For this review, take the finished solid that the model builds, in its own axes (mm). A direction names the side the tool comes from. Give positions to 0.01 mm unless a question says otherwise; leave off trailing zeros. Order: outer loops, then holes, each group sorted by start corner. A loop starts at its lowest first (then second) coordinate and runs counter-clockwise, first axis right, second up. Notation, with made-up numbers: (-27, 76.25) - (-9, 76.25) arc R26 cw to (-9, 92.25) - close; hole circle Ø9 at (22.25, -23). An arc over 180 degrees is marked (long way). One line per item, written item: value.
```python
from build123d import *

# Parameters (mm, degrees)
BASE_PLATE_DEPTH                      = 18
BASE_CORNERS_AND_MOUNTING_HOLES_DEPTH = 36
BASE_RELIEF_SKETCH_R                  = 6
BASE_RELIEF_CUT_DEPTH                 = 36
SUPPORT_UPRIGHT_DEPTH                 = 34
UPRIGHT_TAPER_CUT_DEPTH               = 87.764047854
BEARING_SEAT_CUT_DEPTH                = 12


with BuildPart() as part:
    # Base Plate Profile → Base Plate (new, symmetric)
    with BuildSketch(Plane.XY):
        Polygon((0, 0), (50, 0), (50, 12), (-50, 12), (-50, 0), align=None)
    extrude(amount=BASE_PLATE_DEPTH, both=True)

    # Base Corners and Holes Sketch → Base Corners and Mounting Holes (cut)
    with BuildSketch(Plane(origin=(0, 12, 0), x_dir=(1, 0, 0), z_dir=(0, 1, 0))):
        with BuildLine():
            Line((-50, -14), (-50, -18))
            Line((-50, -18), (-46, -18))
            ThreePointArc((-46, -18), (-48.828427125, -16.828427125), (-50, -14))
        make_face()
        with BuildLine():
            Line((50, -14), (50, -18))
            Line((50, -18), (46, -18))
            ThreePointArc((46, -18), (48.828427125, -16.828427125), (50, -14))
        make_face()
        with BuildLine():
            Line((50, 14), (50, 18))
            Line((50, 18), (46, 18))
            ThreePointArc((46, 18), (48.828427125, 16.828427125), (50, 14))
        make_face()
        with BuildLine():
            Line((-50, 18), (-46, 18))
            ThreePointArc((-46, 18), (-48.828427125, 16.828427125), (-50, 14))
            Line((-50, 14), (-50, 18))
        make_face()
    extrude(amount=-BASE_CORNERS_AND_MOUNTING_HOLES_DEPTH, mode=Mode.SUBTRACT)

    # Base Relief Sketch → Base Relief Cut (cut)
    with BuildSketch(Plane(origin=(0, 12, 0), x_dir=(1, 0, 0), z_dir=(0, 1, 0))):
        with Locations(Location((-36, 0, 0), (0, 0, 180))):
            Circle(BASE_RELIEF_SKETCH_R)
        with Locations(Location((36, 0, 0), (0, 0, 270))):
            Circle(BASE_RELIEF_SKETCH_R)
    extrude(amount=-BASE_RELIEF_CUT_DEPTH, mode=Mode.SUBTRACT)

    # Upright Profile → Support Upright (add)
    with BuildSketch(Plane.XY.offset(18)):
        with BuildLine():
            Line((8, 39.150951317), (8, 48))
            Line((8, 48), (20, 48))
            Line((20, 48), (20, 12))
            Line((20, 12), (-20, 12))
            Line((-20, 12), (-20, 48))
            Line((-20, 48), (-8, 48))
            Line((-8, 48), (-8, 39.150951317))
            ThreePointArc((-8, 39.150951317), (0, 31.150951317), (8, 39.150951317))
        make_face()
    extrude(amount=-SUPPORT_UPRIGHT_DEPTH)

    # Upright Taper Sketch → Upright Taper Cut (cut, through all)
    with BuildSketch(Plane.ZY.offset(20)):
        Polygon((-8, 48), (18, 48), (18, 12), (16, 12), align=None)
    extrude(amount=-UPRIGHT_TAPER_CUT_DEPTH, mode=Mode.SUBTRACT)

    # Bearing Seat Sketch → Bearing Seat Cut (cut, symmetric)
    with BuildSketch(Plane(origin=(0, 0, 0), x_dir=(0, 0, -1), z_dir=(1, 0, 0))):
        Polygon((8, 48), (8, 12), (-16, 12), align=None)
    extrude(amount=BEARING_SEAT_CUT_DEPTH, both=True, mode=Mode.SUBTRACT)


solid = part.part
```
(1) Take a section at D-D (z = -12). Write out the cut boundary in (x, y), then the cut area to 3 significant figures.
Answers below:
outline: (-50, 0) - (50, 0) - (50, 12) - (20, 12) - (20, 48) - (8, 48) - (8, 39.15) arc R8 cw to (-8, 39.15) - (-8, 48) - (-20, 48) - (-20, 12) - (-50, 12) - close
area: 2,400 mm^2
(2) For P1, Ø12, axis at y = 38.5, z = 0, coming from the -X side; P2, Ø7, axis at x = 36, z = 0, coming from the +Y side; P3, Ø9, axis at y = 41.5, z = -10, coming from the +X side; P4, Ø1, axis at x = -6, y = 20, coming from the -Z side, all flat-tipped, find the tip position at first contact; note any pin that passes through.
Answers below:
P1: stops at x = -20
P2: passes through
P3: stops at x = 20
P4: stops at z = -16
(3) Take a section at C-C (y = 15). Write out the cut boundary in (x, z), then the cut area to 3 significant figures.
Answers below:
outline: (-20, -16) - (20, -16) - (20, 14) - (12, 14) - (12, -8) - (-12, -8) - (-12, 14) - (-20, 14) - close
area: 672 mm^2
(4) Take a section at B-B (x = 36). Write out the cut boundary in (y, z).
Answers below:
outline: (0, -18) - (12, -18) - (12, -6) - (0, -6) - close; (0, 6) - (12, 6) - (12, 18) - (0, 18) - close
(5) Wall thickness on line 1 (Z direction, x = -36, y = 4); line 2 (X direction, y = 20, z = -7); line 3 (X direction, y = 39.5, z = -12): over which ranges is each line inside the solid? List them lowest first. Write a range as from..to.
Answers below:
line 1: z = -18..-6, 6..18
line 2: x = -20..-12, 12..20
line 3: x = -20..-8, 8..20
(6) Machinability: for faces 1 (the face through (-8, 44, -12)), 2 (the face through (20, 26, -3)), 3 (the face through (-20, 26, -3)), 4 (the face through (12, 22, -2)), 5 (the face through (0, 30, -16)), which of the approach directions +Z, -Z, +X, -X, +Y, -Y give a long, thin tool a straight path to every point of the face, cutting with its end or side? Answer none if there is none.
Answers below:
face 1: +Z, -Z, +Y
face 2: +Z, -Z, +X, +Y
face 3: +Z, -Z, -X, +Y
face 4: +Z, +Y
face 5: -Z, +X, -X, +Y
(7) Take a section at A-A (z = 0). Write out the cut boundary in (x, y), then the cut area to 3 significant figures.
Answers below:
outline: (-50, 0) - (-42, 0) - (-42, 12) - (-50, 12) - close; (-30, 0) - (30, 0) - (30, 12) - (20, 12) - (20, 36) - (12, 36) - (12, 12) - (-12, 12) - (-12, 36) - (-20, 36) - (-20, 12) - (-30, 12) - close; (42, 0) - (50, 0) - (50, 12) - (42, 12) - close
area: 1,300 mm^2
